from build123d import *

# Parameters (mm, degrees)
SKETCH1_W           = 110.8
SKETCH1_H           = 40
BOSS_EXTRUDE1_DEPTH = 40
SKETCH2_R           = 15
BOSS_EXTRUDE2_DEPTH = 2.6
SKETCH3_R           = 4
BOSS_EXTRUDE3_DEPTH = 23.8
SKETCH4_R           = 10
CUT_EXTRUDE1_DEPTH  = 105.8
CIRPATTERN1_COUNT   = 4


with BuildPart() as part:
    # Sketch1 → Boss-Extrude1 (new body)
    with BuildSketch(Plane.XY):
        Rectangle(SKETCH1_W, SKETCH1_H)
    extrude(amount=BOSS_EXTRUDE1_DEPTH)

    # Sketch2 → Boss-Extrude2 (add)
    with BuildSketch(Plane.ZY.offset(55.4)):
        with Locations(Location((20, 0, 0), (0, 0, 90))):
            Circle(SKETCH2_R)
    extrude(amount=BOSS_EXTRUDE2_DEPTH)

    # Sketch3 → Boss-Extrude3 (add)
    with BuildSketch(Plane.ZY.offset(58)):
        with Locations(Location((20, 0, 0), (0, 0, 270))):
            Circle(SKETCH3_R)
    extrude(amount=BOSS_EXTRUDE3_DEPTH)

    # Sketch4 → Cut-Extrude1 (cut)
    with BuildSketch(Plane(origin=(55.4, 0, 0), x_dir=(0, 0, -1), z_dir=(1, 0, 0))):
        with Locations((-40, 20)):
            Circle(SKETCH4_R)
        with Locations((0, 20)):
            Circle(SKETCH4_R)
        with Locations((-40, -20)):
            Circle(SKETCH4_R)
        with Locations((0, -20)):
            Circle(SKETCH4_R)
    extrude(amount=-CUT_EXTRUDE1_DEPTH, mode=Mode.SUBTRACT)

    # Sketch5 → M4 Clearance Hole1 (revolve, cut)
    with BuildSketch(Plane(origin=(-55.4, 15.909902577, 4.090097423), x_dir=(0, 0, 1), z_dir=(0, 1, 0))):
        Polygon((0, 0), (0, 258.851936393), (2.25, 257.5), (2.25, 0), align=None)
    m4_clearance_hole1 = revolve(axis=Axis((-61.75, 15.909902577, 4.090097423), (1, 0, 0)), mode=Mode.SUBTRACT)

    # CirPattern1: M4 Clearance Hole1 ×4 about axis
    cirpattern1_axis = Axis((0, 0, 20), (1, 0, 0))
    for i in range(1, CIRPATTERN1_COUNT):
        add(m4_clearance_hole1.rotate(cirpattern1_axis, i * 360 / CIRPATTERN1_COUNT), mode=Mode.SUBTRACT)


solid = part.part
Can you work these out from the model? Positions are in its coordinate system, mm. A direction names the side the tool comes from. Coordinates: 2 decimals unless noted, no trailing zeros. Loops run counter-clockwise (first coordinate to the right, second up) from the corner with the lowest first, then second, coordinate; pieces in that order, holes last. Notation, with made-up numbers: (64.25, 46) - (95.25, 46) arc R22 ccw to (95.25, 75) - close; hole circle Ø6 at (26, -16). An arc over 180 degrees is marked (long way). Answer as a JSON object with one key per item and string values. Group by question number.
Item 1: If we section it at C-C (x = -12): List the corners of the cut face in (y, z) for me, plus the area to 3 significant figures.
Item 2: If we section it at A-A (z = 20): List the corners of the cut face in (x, y) for me.
Item 3: If I drill on L1, parallel to X at y = -1.5, z = 15.5; L2, parallel to X at y = -9, z = 33; L3, parallel to Y at x = -71, z = 22, over which ranges is the centre line in solid material (lowest first)? Write a range as from..to.
Item 4: On a 3-axis mill with a long thin cutter (end or side, diameter ignored), from which of +Z, -Z, +X, -X, +Y, -Y can I reach the whole of each face in a straight line? I mean faces 1 (the face through (-56.682, -3.252, 34.643)), 2 (the face through (-50.4, 18.4, 36.2)), 3 (the face through (-50.4, -17.2, 6.2)). Say none if no direction works.
Item 5: If we section it at B-B (y = 0): List the corners of the cut face in (x, z) for me, plus the area to 3 significant figures.
Item 6: If we section it at D-D (z = 11.5): List the corners of the cut face in (x, y) for me, plus the area to 3 significant figures.
Item 7: For pin 1 (7 mm diameter, centred on y = 15.91, z = 4.09, fed in from +X); pin 2 (2 mm diameter, centred on x = 30, z = 35.5, fed in from -Y); pin 3 (1 mm diameter, centred on y = -3, z = 28, fed in from -X); pin 4 (3.5 mm diameter, centred on y = -15.91, z = 35.91, fed in from +X), each with a flat end and sliding along its axis, tell me the tip position at first contact or that it passes through.
Item 8: If we mould it in two halves opening along Y, with no side actions, what happens to faces 4 (the face through (-69.733, 0.521, 23.966)), 5 (the face through (-52.93, 17.57, 34.39)), 6 (the face through (3.24, -12.85, 6.99)), 7 (the face through (-52.935, -15.811, 38.158))? For each: released by +Y, released by -Y, zero draft, split by the parting line, or undercut.
Returned:
{
 "1": {"outline": "(-20, 10) arc R10 cw to (-10, 0) - (10, 0) arc R10 cw to (20, 10) - (20, 30) arc R10 cw to (10, 40) - (-10, 40) arc R10 cw to (-20, 30) - close", "area": "1,290 mm²"},
 "2": {"outline": "(-81.8, -4) - (-58, -4) - (-58, -15) - (-55.4, -15) - (-55.4, -20) - (55.4, -20) - (55.4, 20) - (-55.4, 20) - (-55.4, 15) - (-58, 15) - (-58, 4) - (-81.8, 4) - close"},
 "3": {"L1": "x = -58..55.4", "L2": "x = -55.4..55.4", "L3": "y = -3.46..3.46"},
 "4": {"face 1": "-X", "face 2": "+Z, +X, +Y", "face 3": "-Z, +X, -Y"},
 "5": {"outline": "(-81.8, 16) - (-58, 16) - (-58, 5) - (-55.4, 5) - (-55.4, 0) - (55.4, 0) - (55.4, 40) - (-55.4, 40) - (-55.4, 35) - (-58, 35) - (-58, 24) - (-81.8, 24) - close", "area": "4,700 mm²"},
 "6": {"outline": "(-58, -12.36) - (-55.4, -12.36) - (-55.4, -20) - (55.4, -20) - (55.4, 20) - (-55.4, 20) - (-55.4, 12.36) - (-58, 12.36) - close", "area": "4,500 mm²"},
 "7": {"pin 1": "stops at x = -50.4", "pin 2": "stops at y = -11.65", "pin 3": "stops at x = -58", "pin 4": "passes through"},
 "8": {"face 4": "split by the parting line", "face 5": "undercut", "face 6": "released by -Y", "face 7": "undercut"}
}
